```python
from build123d import *

# Parameters (mm, degrees)
SKETCH1_R               = 2.5
BOSS_EXTRUDE1_DEPTH     = 13.5
SKETCH2_R               = 3
BOSS_EXTRUDE2_DEPTH     = 67
SKETCH3_R               = 2.5
BOSS_EXTRUDE3_DEPTH     = 30.5
SKETCH4_R               = 2
BOSS_EXTRUDE4_DEPTH     = 8
BOSS_EXTRUDE5_START     = 12
SKETCH5_R               = 2
BOSS_EXTRUDE5_DEPTH     = 12
M2_5_TAPPED_HOLE1_D     = 2.05
M2_5_TAPPED_HOLE1_DEPTH = 6.35
M2_5_TAPPED_HOLE1_TIP   = 0.615882135


with BuildPart() as part:
    # Sketch1 → Boss-Extrude1 (new body)
    with BuildSketch(Plane.XY):
        Circle(SKETCH1_R)
    extrude(amount=BOSS_EXTRUDE1_DEPTH)

    # Sketch2 → Boss-Extrude2 (add)
    with BuildSketch(Plane.XY.offset(13.5)):
        Circle(SKETCH2_R)
    extrude(amount=BOSS_EXTRUDE2_DEPTH)

    # Sketch3 → Boss-Extrude3 (add)
    with BuildSketch(Plane.XY.offset(80.5)):
        Circle(SKETCH3_R)
    extrude(amount=BOSS_EXTRUDE3_DEPTH)

    # Sketch4 → Boss-Extrude4 (add)
    with BuildSketch(Plane.XY.offset(111)):
        Circle(SKETCH4_R)
    extrude(amount=BOSS_EXTRUDE4_DEPTH)

    # Sketch5 → Boss-Extrude5 (add)
    with BuildSketch(Plane(origin=(0, 0, 0), x_dir=(-1, 0, 0), z_dir=(0, 0, -1)).offset(BOSS_EXTRUDE5_START)):
        with Locations(Location((0, 0, 0), (0, 0, 180))):
            Circle(SKETCH5_R)
    extrude(amount=-BOSS_EXTRUDE5_DEPTH)

    # M2.5 Tapped Hole1
    with Locations(Plane.XY.offset(119)):
        with Locations((0, 0)):
            Hole(M2_5_TAPPED_HOLE1_D / 2, depth=M2_5_TAPPED_HOLE1_DEPTH)
            with Locations((0, 0, -(M2_5_TAPPED_HOLE1_DEPTH + M2_5_TAPPED_HOLE1_TIP / 2))):  # 118° drill point
                Cone(0, M2_5_TAPPED_HOLE1_D / 2, M2_5_TAPPED_HOLE1_TIP, mode=Mode.SUBTRACT)


solid = part.part
```
The listing builds one solid part. Answer for the finished solid, in the listing's coordinates (mm). A direction names the side the tool comes from. Give positions to 0.01 mm unless a question says otherwise; leave off trailing zeros. Write each loop counter-clockwise with the first axis right and the second up, starting at its lowest first coordinate (ties: lowest second). Pieces come first, ordered by that corner, then holes. Notation, with made-up numbers: (-26, 75) - (25, 75) arc R23 cw to (25, 113) - close; hole circle Ø4 at (58.25, 62). An arc over 180 degrees is marked (long way). Use one line per item in the form item = value. Start each with the question number.
1) Find section A-A on z = 66.5. Determine the outline of the cut face in (x, y), plus the area to 3 significant figures.
2) A tool of negligible diameter and unlimited length cuts with its end or side. For faces 4 (the face through (0.133, 1.016, 115.781)), 5 (the face through (0, 2, -6)), 6 (the face through (0, 0, -12)), from which of +Z, -Z, +X, -X, +Y, -Y can it reach the whole face along a straight path? Write none if from no direction.
3) The mould has two halves that part along X. Classify faces 1 (the face through (-2, 2, 80.5)), 2 (the face through (-0.04, -0.17, 112.14)), 3 (the face through (-0.54, -2.44, 95.54)): pulls with the +X half, pulls with the -X half, needs draft (parallel to the pull), parting line crosses it, or undercut.
4) Find section B-B on z = -2.5. Determine the outline of the cut face in (x, y), plus the area to 3 significant figures.
5) Flat-ended cylindrical pins translate along their axes: pin 1 Ø1.5 at (x, y) = (0, 0) entering from +Z; pin 2 Ø3 at (y, z) = (-2, 43) entering from +X; pin 3 Ø1 at (x, z) = (1, 95.5) entering from -Y; pin 4 Ø2 at (x, y) = (1, -2) entering from -Z. Find the tip coordinate at first contact, or state that the pin passes through.
6) Consider line 1 along Y through (x, z) = (0, 115.5) (3 decimals); line 2 along Z through (x, y) = (0.65, -2.1); line 3 along Z through (x, y) = (-1.5, -2.15). Determine where each line is inside the solid, lowest interval first. Write a range as from..to.
Geometry results:
q1.outline = circle Ø6 at (0, 0)
q1.area = 28.3 mm2
q2.face_4 = +Z
q2.face_5 = -Z
q2.face_6 = -Z, +X, -X, +Y, -Y
q3.face_1 = needs draft
q3.face_2 = undercut
q3.face_3 = parting line crosses it
q4.outline = circle Ø4 at (0, 0)
q4.area = 12.6 mm2
q5.pin_1 = 112.48
q5.pin_2 = 2.96
q5.pin_3 = -2.45
q5.pin_4 = -12
q6.line_1 = -2..-1.025, 1.025..2
q6.line_2 = 0..111
q6.line_3 = 13.5..80.5
